```python
from build123d import *

# Parameters (mm, degrees)
SKETCH_1_W                   = 60
SKETCH_1_H                   = 120
EXTRUDE_1_DEPTH              = 2
SKETCH_2_W                   = 36
SKETCH_2_H                   = 76
CUT_EXTRUDE_1_DEPTH          = 68.201190466
SKETCH_3_W                   = 40.2
SKETCH_3_H                   = 80.2
CUT_EXTRUDE_2_DEPTH          = 1
HOLE_WIZARD_3_0_3_1_D        = 3
HOLE_WIZARD_3_0_3_1_DEPTH    = 1
FILLET_1_R                   = 3
HOLE_WIZARD_M2_1_D           = 2.4
HOLE_WIZARD_M2_1_CBORE_D     = 4.4
HOLE_WIZARD_M2_1_CBORE_DEPTH = 2.4
HOLE_WIZARD_M3_1_D           = 2.5


with BuildPart() as part:
    # 草图1 → 凸台-拉伸1 (new, symmetric)
    with BuildSketch(Plane.XY):
        Rectangle(SKETCH_1_W, SKETCH_1_H)
    extrude(amount=EXTRUDE_1_DEPTH, both=True)

    # 草图2 → 切除-拉伸1 (cut, through all)
    with BuildSketch(Plane.XY.offset(2)):
        with Locations((-2, 0)):
            Rectangle(SKETCH_2_W, SKETCH_2_H)
    extrude(amount=-CUT_EXTRUDE_1_DEPTH, mode=Mode.SUBTRACT)

    # 草图3 → 切除-拉伸2 (cut)
    with BuildSketch(Plane.XY.offset(2)):
        with Locations((-2, 0)):
            Rectangle(SKETCH_3_W, SKETCH_3_H)
    extrude(amount=-CUT_EXTRUDE_2_DEPTH, mode=Mode.SUBTRACT)

    # Ø3.0 (3) 直径孔1
    with Locations(Plane.XY.offset(2)):
        with Locations((-20.6, 40.1), (16.6, 40.1), (16.6, -40.1), (-20.6, -40.1)):
            Hole(HOLE_WIZARD_3_0_3_1_D / 2, depth=HOLE_WIZARD_3_0_3_1_DEPTH)

    # 圆角1
    fillet_1_edges = [part.edges().sort_by_distance(p)[0] for p in [
        (-20, -38, -0.5),
        (-20, 38, -0.5),
        (16, 38, -0.5),
        (16, -38, -0.5),
    ]]
    fillet(fillet_1_edges, radius=FILLET_1_R)

    # M2 六角凹头螺钉的柱形沉头孔1 (through all)
    with Locations(Plane.XY.offset(2)):
        with Locations((-28, 0), (28, 0), (-15, 58), (15, 58), (-28, 35), (28, 35), (-28, -35), (28, -35), (-15, -58), (15, -58)):
            CounterBoreHole(HOLE_WIZARD_M2_1_D / 2, HOLE_WIZARD_M2_1_CBORE_D / 2, HOLE_WIZARD_M2_1_CBORE_DEPTH)

    # M3 螺纹孔1 (through all)
    with Locations(Plane.XY.offset(2)):
        with Locations((-22.5, 56), (22.5, 56), (-26, 25), (26, 25), (26, -25), (-26, -25), (22.5, -56), (-22.5, -56)):
            Hole(HOLE_WIZARD_M3_1_D / 2)


solid = part.part
```
Could you check a few things on this model? Use its own coordinates, in mm. A direction names the side the tool comes from. Give positions to 0.01 mm unless a question says otherwise; leave off trailing zeros. Loops run counter-clockwise (first coordinate to the right, second up) from the corner with the lowest first, then second, coordinate; pieces in that order, holes last. Notation, with made-up numbers: (70.5, 63) - (118.5, 63) arc R24 cw to (118.5, 86) - close; hole circle Ø2 at (6.5, 63). An arc over 180 degrees is marked (long way). Answer in a Markdown table with one row per item. Add a question column.
Q1. We'd pull the mould along Y, two halves only. Please class faces 3 (the face through (-27.155, -25.479, -0.028)), 4 (the face through (30, -1, -1)): +Y half, -Y half, draft (parallel to the pull), parting line (faces both ways), or undercut.
Q2. If we section it at C-C (x = -7): List the corners of the cut face in (y, z) for me, plus the area to 3 significant figures.
Q3. If we section it at B-B (y = 10): List the corners of the cut face in (x, z) for me, plus the area to 3 significant figures.
Q4. Which directions (+Z, -Z, +X, -X, +Y, -Y) give clear straight access to the entire face, cutting with the end or side of a thin tool? Please do faces 1 (the face through (15.14, 37.1, -0.52)), 2 (the face through (-25.8, -35.08, 0.82)).
Q5. Please list where these lines run through material, in increasing order: L1, parallel to X at y = 58, z = 0.2; L2, parallel to Y at x = 28, z = -1.05; L3, parallel to Y at x = 22.5, z = 0.6. Write a range as from..to.
Q6. For pin 1 (2 mm diameter, centred on x = -20, y = 20, fed in from +Z); pin 2 (2 mm diameter, centred on x = -15.5, y = -59, fed in from +Z); pin 3 (2 mm diameter, centred on x = -15, y = -58, fed in from +Z), each with a flat end and sliding along its axis, tell me the tip position at first contact or that it passes through.
Q7. If we section it at A-A (x = 22.5): List the corners of the cut face in (y, z) for me, plus the area to 3 significant figures.
The answers:
| question | item | result |
|---|---|---|
| 1 | face 3 | undercut |
| 1 | face 4 | draft |
| 2 | outline | (-60, -2) - (-38, -2) - (-38, 1) - (-40.1, 1) - (-40.1, 2) - (-60, 2) - close; (38, -2) - (60, -2) - (60, 2) - (40.1, 2) - (40.1, 1) - (38, 1) - close |
| 2 | area | 172 mm^2 |
| 3 | outline | (-30, -2) - (-20, -2) - (-20, 1) - (-22.1, 1) - (-22.1, 2) - (-30, 2) - close; (16, -2) - (30, -2) - (30, 2) - (18.1, 2) - (18.1, 1) - (16, 1) - close |
| 3 | area | 91.8 mm^2 |
| 4 | face 1 | +Z, -Z |
| 4 | face 2 | +Z |
| 5 | L1 | x = -30..-17.2, -12.8..12.8, 17.2..30 |
| 5 | L2 | y = -60..-36.2, -33.8..-1.2, 1.2..33.8, 36.2..60 |
| 5 | L3 | y = -60..-57.25, -54.75..54.75, 57.25..60 |
| 6 | pin 1 | stops at z = 1 |
| 6 | pin 2 | stops at z = -0.4 |
| 6 | pin 3 | passes through |
| 7 | outline | (-60, -2) - (-57.25, -2) - (-57.25, 2) - (-60, 2) - close; (-54.75, -2) - (54.75, -2) - (54.75, 2) - (-54.75, 2) - close; (57.25, -2) - (60, -2) - (60, 2) - (57.25, 2) - close |
| 7 | area | 460 mm^2 |
